Check sheet for the modelled part. Datum: model origin and axes. Units: mm. A direction names the side the tool comes from. Round coordinates to 2 decimals unless told otherwise and drop trailing zeros. Write each loop counter-clockwise with the first axis right and the second up, starting at its lowest first coordinate (ties: lowest second). Pieces come first, ordered by that corner, then holes. Notation, with made-up numbers: (86.25, 48) -> (136.25, 48) arc R22 ccw to (136.25, 63) -> close; hole circle Ø6 at (16, -11). An arc over 180 degrees is marked (long way). One line per item, written item: value. Start each with the question number.
```python
from build123d import *

# Parameters (mm, degrees)
SHANK_PROFILE_75_R   = 37.5
SHANK_75_DEPTH       = 115
HEAD_PROFILE_100_R   = 50
FORK_HEAD_100_DEPTH  = 70
FLAT_FACE_CUT_DEPTH  = 230
FORK_SLOT_PROFILE_R  = 16
FORK_SLOT_PROFILE_W  = 50
FORK_SLOT_PROFILE_H  = 62.840020357
FORK_SLOT_CUT_DEPTH  = 230
CROSS_HOLE_PROFILE_W = 75
CROSS_HOLE_PROFILE_H = 40
CROSS_HOLE_CUT_DEPTH = 25


with BuildPart() as part:
    # Shank Profile Ø75 → Shank Ø75 (new body)
    with BuildSketch(Plane(origin=(0, 0, 0), x_dir=(1, 0, 0), z_dir=(0, 1, 0))):
        with Locations(Location((0, 0, 0), (0, 0, 270))):
            Circle(SHANK_PROFILE_75_R)
    extrude(amount=SHANK_75_DEPTH)

    # Head Profile Ø100 → Fork Head Ø100 (add)
    with BuildSketch(Plane(origin=(0, 115, 0), x_dir=(1, 0, 0), z_dir=(0, 1, 0))):
        with Locations(Location((0, 0, 0), (0, 0, 270))):
            Circle(HEAD_PROFILE_100_R)
    extrude(amount=FORK_HEAD_100_DEPTH)

    # Flat Face Profile → Flat Face Cut (cut)
    with BuildSketch(Plane(origin=(0, 185, 0), x_dir=(1, 0, 0), z_dir=(0, 1, 0))):
        Polygon((-81.032063785, -19), (77.121249896, -19), (5.631572001, -69.155704166), align=None)
    extrude(amount=-FLAT_FACE_CUT_DEPTH, mode=Mode.SUBTRACT)

    # Fork Slot Profile → Fork Slot Cut (cut)
    with BuildSketch(Plane.XY.offset(19)):
        with Locations((0, 73)):
            Circle(FORK_SLOT_PROFILE_R)
        with Locations((0, 168.420010179)):
            Rectangle(FORK_SLOT_PROFILE_W, FORK_SLOT_PROFILE_H)
    extrude(amount=-FORK_SLOT_CUT_DEPTH, mode=Mode.SUBTRACT)

    # Cross Hole Profile → Cross Hole Cut (cut)
    with BuildSketch(Plane.XY.offset(19)):
        with Locations((0, 20)):
            Rectangle(CROSS_HOLE_PROFILE_W, CROSS_HOLE_PROFILE_H)
    extrude(amount=-CROSS_HOLE_CUT_DEPTH, mode=Mode.SUBTRACT)


solid = part.part
```
1. Material ranges on probe 1 along X at (y, z) = (73, 1); probe 2 along Y at (x, z) = (0, -4); probe 3 along Y at (x, z) = (-17.5, 16), recorded low to high.
2. Cross-section at B-B (z = 0). Record the cut outline in (x, y), plus the area to 3 significant figures.
3. Release check for a two-part mould opening along X. For faces 1 (the face through (1.103, 56.695, -37.484)), 2 (the face through (-25, 161, -12)), 3 (the face through (-35, 185, -6)) record: +X half, -X half, draft (parallel to the pull), parting line (faces both ways), or undercut.
4. Depth check by flat-ended pin: pin 1 Ø12 at (x, y) = (9.5, 47) entering from -Z; pin 2 Ø25 at (x, z) = (7, -27.5) entering from +Y; pin 3 Ø12 at (x, z) = (3, 3.5) entering from -Y. Enter the tip coordinate at first touch or a pass-through.
5. Cross-section at C-C (y = 146). Record the cut outline in (x, z), plus the area to 3 significant figures.
6. Cross-section at D-D (x = 40). Record the cut outline in (y, z).
7. Cross-section at A-A (x = 0). Record the cut outline in (y, z).
8. Access from +Z, -Z, +X, -X, +Y, -Y to the whole of each face (thin tool, end or side, straight path). Record for faces 4 (the face through (-1, 40, 7)), 5 (the face through (0, 137, -15)), 6 (the face through (1.37, 133.95, -49.98)).
Working result:
1. probe 1: x = -37.49 to -16, 16 to 37.49
1. probe 2: y = 40 to 57, 89 to 137
1. probe 3: y = 40 to 137
2. outline: (-50, 115) -> (-37.5, 115) -> (-37.5, 40) -> (37.5, 40) -> (37.5, 115) -> (50, 115) -> (50, 185) -> (25, 185) -> (25, 137) -> (-25, 137) -> (-25, 185) -> (-50, 185) -> close; hole circle Ø32 at (0, 73)
2. area: 9,420 mm^2
3. face 1: parting line
3. face 2: undercut
3. face 3: draft
4. pin 1: stops at z = -37.34
4. pin 2: stops at y = 137
4. pin 3: stops at y = 40
5. outline: (-46.25, 19) arc R50 ccw to (-25, -43.3) -> (-25, 19) -> close; (25, -43.3) arc R50 ccw to (46.25, 19) -> (25, 19) -> close
5. area: 2,440 mm^2
6. outline: (115, -30) -> (185, -30) -> (185, 19) -> (115, 19) -> close
7. outline: (0, -37.5) -> (57, -37.5) -> (57, 19) -> (40, 19) -> (40, -6) -> (0, -6) -> close; (89, -37.5) -> (115, -37.5) -> (115, -50) -> (137, -50) -> (137, 19) -> (89, 19) -> close
8. face 4: +Z, +X, -X, -Y
8. face 5: +Z, -Z, +Y
8. face 6: +Y, -Y
